The listing builds one solid part. Answer for the finished solid, in the listing's coordinates (mm). Round coordinates to 2 decimals unless told otherwise and drop trailing zeros. Write each loop counter-clockwise with the first axis right and the second up, starting at its lowest first coordinate (ties: lowest second). Pieces come first, ordered by that corner, then holes. Notation, with made-up numbers: M 49,76 L 106,76 A9 cw 106,89 Z; hole C 73,32.5 d10. An arc over 180 degrees is marked long. Answer as CSV lines item,"result". Start each with the question number.
from build123d import *

# Parameters (mm, degrees)
SKETCH_1_W          = 90
SKETCH_1_H          = 20
EXTRUDE_1_DEPTH     = 1.5
SKETCH_2_R          = 2.5
CUT_EXTRUDE_1_DEPTH = 47.122120506
FILLET_1_R          = 2


with BuildPart() as part:
    # 草图1 → 凸台-拉伸1 (new body)
    with BuildSketch(Plane(origin=(0, 0, 0), x_dir=(1, 0, 0), z_dir=(0, 1, 0))):
        Rectangle(SKETCH_1_W, SKETCH_1_H)
    extrude(amount=EXTRUDE_1_DEPTH)

    # 草图2 → 切除-拉伸1 (cut, through all)
    with BuildSketch(Plane(origin=(0, 1.5, 0), x_dir=(1, 0, 0), z_dir=(0, 1, 0))):
        with Locations(Location((-39, 0, 0), (0, 0, 270))):
            Circle(SKETCH_2_R)
        with Locations(Location((39, 0, 0), (0, 0, 270))):
            Circle(SKETCH_2_R)
    extrude(amount=-CUT_EXTRUDE_1_DEPTH, mode=Mode.SUBTRACT)

    # 圆角1
    fillet_1_edges = [part.edges().sort_by_distance(p)[0] for p in [
        (45, 0.75, 10),
        (-45, 0.75, 10),
        (-45, 0.75, -10),
        (45, 0.75, -10),
    ]]
    fillet(fillet_1_edges, radius=FILLET_1_R)


solid = part.part
Q1. Find section B-B (y = 0.7). Determine the outline of the cut face in (x, z).
Q2. Find section C-C (x = -39). Determine the outline of the cut face in (y, z).
Q3. This flat-tipped pin is pushed along its axis until it touches: P1, Ø6.5, axis at x = -39, z = 0, coming from the +Y side. Where does it stop, or does it pass through?
Q4. Straight lines are drawn through the part: L1, parallel to X at y = 1, z = 0; L2, parallel to X at y = 0.25, z = 2.25. For each, find the intervals that lie inside material, in ascending order.
Q5. Find section A-A (z = 0). Determine the outline of the cut face in (x, y), plus the area to 3 significant figures.
Q6. The mould has two halves that part along Z. Classify faces 1 (the face through (45, 1, 0)), 2 (the face through (-41.44, 0.76, -0.54)), 3 (the face through (44.4, 0.76, -9.43)): +Z half, -Z half, draft (parallel to the pull), parting line (faces both ways), or undercut.
Reported:
1,outline,"M -45,-8 A2 ccw -43,-10 L 43,-10 A2 ccw 45,-8 L 45,8 A2 ccw 43,10 L -43,10 A2 ccw -45,8 Z; hole C -39,0 d5; hole C 39,0 d5"
2,outline,"M 0,-10 L 1.5,-10 L 1.5,-2.5 L 0,-2.5 Z; M 0,2.5 L 1.5,2.5 L 1.5,10 L 0,10 Z"
3,P1,"stops at y = 1.5"
4,L1,"x = -45 to -41.5, -36.5 to 36.5, 41.5 to 45"
4,L2,"x = -45 to -40.09, -37.91 to 37.91, 40.09 to 45"
5,outline,"M -45,0 L -41.5,0 L -41.5,1.5 L -45,1.5 Z; M -36.5,0 L 36.5,0 L 36.5,1.5 L -36.5,1.5 Z; M 41.5,0 L 45,0 L 45,1.5 L 41.5,1.5 Z"
5,area,"120 mm2"
6,face 1,"draft"
6,face 2,"undercut"
6,face 3,"-Z half"
